Part model, mm, in its own coordinate system. Face numbers are marked on the shaded views. A direction names the side the tool comes from. Give positions to 0.01 mm unless a question says otherwise; leave off trailing zeros. Order: outer loops, then holes, each group sorted by start corner. A loop starts at its lowest first (then second) coordinate and runs counter-clockwise, first axis right, second up. Notation, with made-up numbers: (-14.5, 88.5) - (12.5, 88.5) arc R23 ccw to (12.5, 116.5) - close; hole circle Ø6 at (60.5, -11). An arc over 180 degrees is marked (long way). Use one line per item in the form item = value. Start each with the question number.
1. Drill centre lines: line 1 (Y direction, x = 46.48, z = 2.5); line 2 (Z direction, x = -48.5, y = 37.5); line 3 (X direction, y = 20, z = -7). Where is each one in solid material? Low to high.
2. Band-saw the part on B-B, the plane x = 46.48. List the corners of the cut face in (y, z), plus the area to 3 significant figures.
3. Pin check, flat tips, straight feed: P1, Ø12, axis at x = -1, y = 7.5, coming from the +Z side; P2, Ø14.5, axis at x = -0.5, y = 0, coming from the -Z side; P3, Ø2, axis at x = 28, z = -8, coming from the +Y side. Stop position of each tip, or through.
4. Band-saw the part on A-A, the plane z = -24. List the corners of the cut face in (x, y), plus the area to 3 significant figures.
5. Band-saw the part on C-C, the plane y = -11. List the corners of the cut face in (x, z).
6. Tool access for the marked faces 1, 2 and 3: list every direction of +Z, -Z, +X, -X, +Y, -Y with a clear straight run to the whole face (end or side of a thin tool).
7. Band-saw the part on D-D, the plane y = 20. List the corners of the cut face in (x, z).
8. Pull direction X, two halves, no side cores. Call the marked faces 4, 5, 6 and 7: +X half, -X half, draft (parallel to the pull), parting line (faces both ways), or undercut.
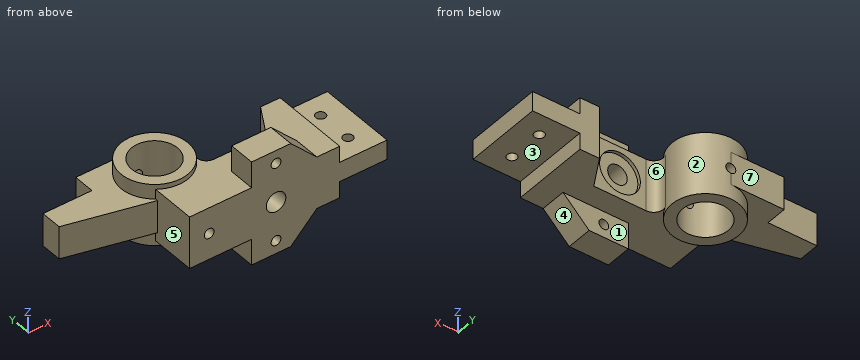
from build123d import *

# Parameters (mm, degrees)
BASE_BLOCK_SKETCH_W                = 121
BASE_BLOCK_SKETCH_H                = 48
BASE_BLOCK_121X48_DEPTH            = 16
BASE_STEP_SKETCH_W                 = 10
BASE_STEP_SKETCH_H                 = 48
BASE_STEP_CUT_DEPTH                = 29
ANGLED_RELIEF_CUT_30DEG_DEPTH      = 73.527580961
ANGLED_RELIEF_CUT_30DEG_DEPTH_BACK = 73.527580961
PIVOT_BOSS_SKETCH_R                = 20.5
PIVOT_BOSS_44_DEPTH                = 19
PIVOT_BOSS_FILLET_R6_R             = 6
CLAMP_TAB_DEPTH                    = 10
TAB_PIN_HOLE_6_DEPTH               = 120.841457826
TAB_PIN_HOLE_6_DEPTH_BACK          = 120.841457826
TAB_PIN_HOLE_SKETCH_R              = 3
PIVOT_BORE_28_DEPTH                = 125.277813908
PIVOT_BORE_28_DEPTH_BACK           = 125.277813908
PIVOT_BORE_SKETCH_R                = 14
COUNTERBORED_HOLE_12_D             = 12
COUNTERBORED_HOLE_12_CBORE_D       = 25
COUNTERBORED_HOLE_12_CBORE_DEPTH   = 2
MOUNTING_FLANGE_SKETCH_R           = 3
MOUNTING_FLANGE_DEPTH              = 16
END_SLOT_CUT_DEPTH                 = 125.277813877
END_SLOT_CUT_DEPTH_BACK            = 125.277813877
END_SLOT_SKETCH_R                  = 3


with BuildPart() as part:
    # Base Block Sketch → Base Block 121x48 (new, symmetric)
    with BuildSketch(Plane.XY):
        Rectangle(BASE_BLOCK_SKETCH_W, BASE_BLOCK_SKETCH_H)
    extrude(amount=BASE_BLOCK_121X48_DEPTH, both=True)

    # Base Step Sketch → Base Step Cut (cut)
    with BuildSketch(Plane(origin=(60.5, 0, 0), x_dir=(0, 0, -1), z_dir=(1, 0, 0))):
        with Locations((-11, 0)):
            Rectangle(BASE_STEP_SKETCH_W, BASE_STEP_SKETCH_H)
        with Locations((11, 0)):
            Rectangle(BASE_STEP_SKETCH_W, BASE_STEP_SKETCH_H)
    extrude(amount=-BASE_STEP_CUT_DEPTH, mode=Mode.SUBTRACT)

    # Angled Relief Sketch → Angled Relief Cut 30deg (cut, two sides: drawn at the far end of the back side and taken through both)
    with BuildSketch(Plane.XY.offset(16).offset(-ANGLED_RELIEF_CUT_30DEG_DEPTH_BACK)):
        Polygon((19.5, 24), (8.530344885, 5), (-40, 5), (-40, 24), align=None)
    extrude(amount=ANGLED_RELIEF_CUT_30DEG_DEPTH + ANGLED_RELIEF_CUT_30DEG_DEPTH_BACK, mode=Mode.SUBTRACT)

    # Pivot Boss Sketch → Pivot Boss Ø44 (add, symmetric)
    with BuildSketch(Plane.XY):
        with Locations((-48.5, 20)):
            Circle(PIVOT_BOSS_SKETCH_R)
    extrude(amount=PIVOT_BOSS_44_DEPTH, both=True)

    # Pivot Boss Fillet R6
    pivot_boss_fillet_r6_edges = [part.edges().sort_by_distance(p)[0] for p in [
        (-34.526811388, 5, 0),
    ]]
    fillet(pivot_boss_fillet_r6_edges, radius=PIVOT_BOSS_FILLET_R6_R)

    # Clamp Tab Sketch → Clamp Tab (add, symmetric)
    with BuildSketch(Plane.XY):
        with BuildLine():
            Line((-48.5, 40.5), (-81.178797502, 40.5))
            Line((-81.178797502, 40.5), (-81.178797502, 27.5))
            Line((-81.178797502, 27.5), (-111.178797502, 27.5))
            Line((-111.178797502, 27.5), (-111.178797502, 14.5))
            Line((-111.178797502, 14.5), (-53.45939886, 0.108937611))
            ThreePointArc((-53.45939886, 0.108937611), (-68.847196109, 22.49832154), (-48.5, 40.5))
        make_face()
    extrude(amount=CLAMP_TAB_DEPTH, both=True)

    # Tab Pin Hole Sketch → Tab Pin Hole Ø6 (cut, two sides: drawn at the far end of the back side and taken through both)
    with BuildSketch(Plane(origin=(0, 0, 0), x_dir=(1, 0, 0), z_dir=(0, 1, 0)).offset(-TAB_PIN_HOLE_6_DEPTH_BACK)):
        with Locations(Location((-48.5, 0, 0), (0, 0, 270))):
            Circle(TAB_PIN_HOLE_SKETCH_R)
    extrude(amount=TAB_PIN_HOLE_6_DEPTH + TAB_PIN_HOLE_6_DEPTH_BACK, mode=Mode.SUBTRACT)

    # Pivot Bore Sketch → Pivot Bore Ø28 (cut, two sides: drawn at the far end of the back side and taken through both)
    with BuildSketch(Plane.XY.offset(19).offset(-PIVOT_BORE_28_DEPTH_BACK)):
        with Locations((-48.5, 20)):
            Circle(PIVOT_BORE_SKETCH_R)
    extrude(amount=PIVOT_BORE_28_DEPTH + PIVOT_BORE_28_DEPTH_BACK, mode=Mode.SUBTRACT)

    # Counterbored Hole Ø12 (through all)
    with Locations(Plane(origin=(0, 5, 0), x_dir=(1, 0, 0), z_dir=(0, 1, 0))):
        with Locations((-7.522383977, 0)):
            CounterBoreHole(COUNTERBORED_HOLE_12_D / 2, COUNTERBORED_HOLE_12_CBORE_D / 2, COUNTERBORED_HOLE_12_CBORE_DEPTH)

    # Mounting Flange Sketch → Mounting Flange (add)
    # profile 1 of 2: a face of its own
    with BuildSketch(Plane.XZ.offset(24)):
        Polygon((-22.5, -16), (-22.5, -32), (1.5, -32), (17.5, -16), align=None)
        with Locations(Location((-7.522383977, -24, 0), (0, 0, 270))):
            Circle(MOUNTING_FLANGE_SKETCH_R, mode=Mode.SUBTRACT)
    # profile 2 of 2: a face of its own
    with BuildSketch(Plane.XZ.offset(24)):
        Polygon((17.5, 16), (-22.5, 16), (-22.5, 32), (1.5, 32), align=None)
        with Locations(Location((-7.522383977, 24, 0), (0, 0, 270))):
            Circle(MOUNTING_FLANGE_SKETCH_R, mode=Mode.SUBTRACT)
    extrude(amount=-MOUNTING_FLANGE_DEPTH)

    # End Slot Sketch → End Slot Cut (cut, two sides: drawn at the far end of the back side and taken through both)
    with BuildSketch(Plane.XY.offset(6).offset(-END_SLOT_CUT_DEPTH_BACK)):
        with Locations((46.48, 11)):
            Circle(END_SLOT_SKETCH_R)
        with Locations((46.48, -11)):
            Circle(END_SLOT_SKETCH_R)
    extrude(amount=END_SLOT_CUT_DEPTH + END_SLOT_CUT_DEPTH_BACK, mode=Mode.SUBTRACT)


solid = part.part
From the geometry:
q1.line_1 = -24 to -14, -8 to 8, 14 to 24
q1.line_2 = -19 to -3, 3 to 19
q1.line_3 = -111.18 to -62.5, -34.5 to -28, 17.19 to 31.5
q2.outline = (-24, -6) - (-14, -6) - (-14, 6) - (-24, 6) - close; (-8, -6) - (8, -6) - (8, 6) - (-8, 6) - close; (14, -6) - (24, -6) - (24, 6) - (14, 6) - close
q2.area = 432 mm²
q3.P1 = 16
q3.P2 = -16
q3.P3 = 24
q4.outline = (-22.5, -24) - (-10.52, -24) - (-10.52, -8) - (-22.5, -8) - close; (-4.52, -24) - (9.5, -24) - (9.5, -8) - (-4.52, -8) - close
q4.area = 416 mm²
q5.outline = (-60.5, -16) - (-22.5, -16) - (-22.5, -32) - (1.5, -32) - (17.5, -16) - (31.5, -16) - (31.5, -6) - (43.48, -6) - (43.48, 6) - (31.5, 6) - (31.5, 16) - (17.5, 16) - (1.5, 32) - (-22.5, 32) - (-22.5, 16) - (-60.5, 16) - close; (49.48, -6) - (60.5, -6) - (60.5, 6) - (49.48, 6) - close; hole circle Ø6 at (-48.5, 0); hole circle Ø12 at (-7.52, 0); hole circle Ø6 at (-7.52, -24); hole circle Ø6 at (-7.52, 24)
q6.face_1 = -Z, +X, -X, +Y
q6.face_2 = none
q6.face_3 = -Z, +X, +Y, -Y
q7.outline = (-111.18, -10) - (-69, -10) - (-69, -19) - (-62.5, -19) - (-62.5, 19) - (-69, 19) - (-69, 10) - (-111.18, 10) - close; (-34.5, -19) - (-28, -19) - (-28, 19) - (-34.5, 19) - close; (17.19, -16) - (31.5, -16) - (31.5, -6) - (60.5, -6) - (60.5, 6) - (31.5, 6) - (31.5, 16) - (17.19, 16) - close
q8.face_4 = +X half
q8.face_5 = -X half
q8.face_6 = undercut
q8.face_7 = draft
